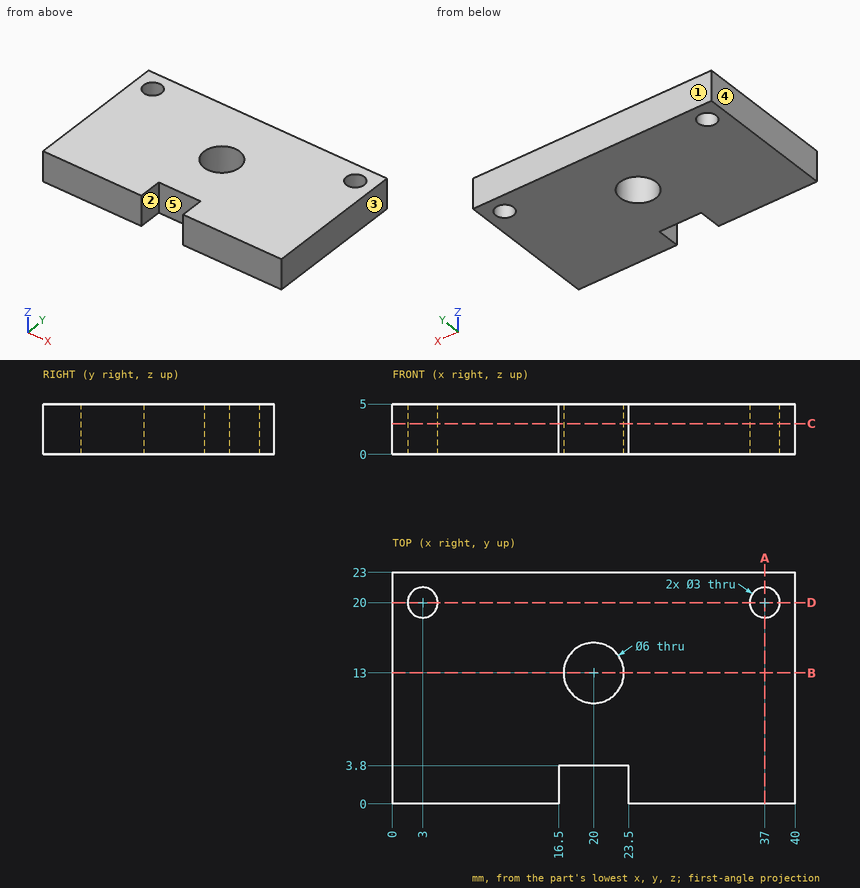
Design review of the part shown in the three views and the two pictorial views. Dimensions are in mm from the part's minimum x, y and z. A direction names the side the tool comes from. Give positions to 0.01 mm unless a question says otherwise; leave off trailing zeros. Loops run counter-clockwise (first coordinate to the right, second up) from the corner with the lowest first, then second, coordinate; pieces in that order, holes last. Notation, with made-up numbers: M -36,36 L -6,36 A18 cw -6,61 Z; hole C -14.5,-23 d8. An arc over 180 degrees is marked long. Answer as a JSON object with one key per item and string values. Group by question number.
Q1. Add section C-C on z = 3.05. Give the boundary of the cut face in (x, y), and give its area (3 significant figures).
Q2. Insertion check: P1, Ø2.5, axis at x = 3, y = 20, coming from the -Z side. The pin has a flat end and moves straight along its axis. Give the tip position at first contact, or say it passes through.
Q3. Mouldability with a two-part tool opening along X and no side actions: class the marked faces 1, 2 and 3 as +X half, -X half, draft (parallel to the pull), parting line (faces both ways), or undercut.
Q4. Tool access review of the marked faces 4 and 5: name each direction out of +Z, -Z, +X, -X, +Y, -Y from which nothing blocks a thin tool from reaching the whole face with its end or side.
Q5. For probe 1 along Y at (x, z) = (20, 3.7); probe 2 along X at (y, z) = (20.25, 0.7); probe 3 along Y at (x, z) = (37, 1.9), list the stretches that pass through material, from the lowest coordinate up. Write a range as [from, to].
Q6. Add section A-A on x = 37. Give the boundary of the cut face in (y, z).
Q7. Add section B-B on y = 13. Give the boundary of the cut face in (x, z), and give its area (3 significant figures).
Q8. Add section D-D on y = 20. Give the boundary of the cut face in (x, z).
Checked values:
{
 "1": {"outline": "M 0,0 L 16.5,0 L 16.5,3.8 L 23.5,3.8 L 23.5,0 L 40,0 L 40,23 L 0,23 Z; hole C 3,20 d3; hole C 20,13 d6; hole C 37,20 d3", "area": "851 mm²"},
 "2": {"P1": "through"},
 "3": {"face 1": "draft", "face 2": "undercut", "face 3": "+X half"},
 "4": {"face 4": "+Z, -Z, -X, +Y, -Y", "face 5": "+Z, -Z, -Y"},
 "5": {"probe 1": "[3.8, 10], [16, 23]", "probe 2": "[0, 1.52], [4.48, 35.52], [38.48, 40]", "probe 3": "[0, 18.5], [21.5, 23]"},
 "6": {"outline": "M 0,0 L 18.5,0 L 18.5,5 L 0,5 Z; M 21.5,0 L 23,0 L 23,5 L 21.5,5 Z"},
 "7": {"outline": "M 0,0 L 17,0 L 17,5 L 0,5 Z; M 23,0 L 40,0 L 40,5 L 23,5 Z", "area": "170 mm²"},
 "8": {"outline": "M 0,0 L 1.5,0 L 1.5,5 L 0,5 Z; M 4.5,0 L 35.5,0 L 35.5,5 L 4.5,5 Z; M 38.5,0 L 40,0 L 40,5 L 38.5,5 Z"}
}
